```python
from build123d import *

# Parameters (mm, degrees)
BASEHEAD_DEPTH = 10.18
SKETCH5_R      = 8
BASEBODY_DEPTH = 35
CHAMFER1_SIZE  = 0.8


with BuildPart() as part:
    # Sketch2 → BaseHead (new body)
    with BuildSketch(Plane(origin=(0, 0, 0), x_dir=(0, 0, -1), z_dir=(1, 0, 0))):
        Polygon((11.835, -6.832940436), (11.835, 6.832940436), (0, 13.665880872), (-11.835, 6.832940436), (-11.835, -6.832940436), (0, -13.665880872), align=None)
    extrude(amount=BASEHEAD_DEPTH)

    # Sketch3 → BearingFace (revolve, cut)
    with BuildSketch(Plane.XY, mode=Mode.PRIVATE) as bearingface_sk:
        Polygon((10.18, 13.665880872), (10.18, 11.245), (9.38, 12.045), (9.38, 13.665880872), align=None)
    revolve(bearingface_sk.sketch.rotate(Axis((-0.957090588, 0, 0), (1, 0, 0)), 90), axis=Axis((-0.957090588, 0, 0), (1, 0, 0)), mode=Mode.SUBTRACT)

    # Sketch4 → HeadChamfer (revolve, cut)
    with BuildSketch(Plane.XY):
        Polygon((0, 13.665880872), (0.66638614, 13.665880872), (0, 11.835), align=None)
    revolve(axis=Axis((-0.493528746, 0, 0), (1, 0, 0)), mode=Mode.SUBTRACT)

    # Sketch5 → BaseBody (add)
    with BuildSketch(Plane(origin=(10.18, 0, 0), x_dir=(0, 0, -1), z_dir=(1, 0, 0))):
        with Locations(Location((0, 0, 0), (0, 0, 180))):
            Circle(SKETCH5_R)
    extrude(amount=BASEBODY_DEPTH)

    # Chamfer1
    chamfer1_edges = [part.edges().sort_by_distance(p)[0] for p in [
        (45.18, 0, -8),
    ]]
    chamfer(chamfer1_edges, length=CHAMFER1_SIZE)


solid = part.part
```
Could you check a few things on this model? Use its own coordinates, in mm. A direction names the side the tool comes from. Give positions to 0.01 mm unless a question says otherwise; leave off trailing zeros. Loops run counter-clockwise (first coordinate to the right, second up) from the corner with the lowest first, then second, coordinate; pieces in that order, holes last. Notation, with made-up numbers: (1.25, 74.25) -> (10.25, 74.25) arc R17 ccw to (10.25, 102.25) -> close; hole circle Ø9 at (27, 85). An arc over 180 degrees is marked (long way). Put each result on its own line as item: value.
(1) I'm going to push flat-ended pins straight in: pin 1 Ø4 at (y, z) = (9, 4.5) entering from +X; pin 2 Ø3 at (x, y) = (20, 5.5) entering from +Z; pin 3 Ø5 at (x, z) = (12, 6) entering from -Y. Where does each tip first touch, or does it pass through?
Computed:
pin 1: x = 10.18
pin 2: z = 6.93
pin 3: y = -10.6
(2) Please list where these lines run through material, in increasing order: probe 1 along X at (y, z) = (-8.25, 2.75); probe 2 along Z at (x, y) = (42, -1.5); probe 3 along Y at (x, z) = (13, -0.75). Write a range as [from, to].
Computed:
probe 1: [0, 10.18]
probe 2: [-7.86, 7.86]
probe 3: [-7.96, 7.96]
(3) Imagine slicing it at A-A on x = 16. Write out the boundary of the cut face in (y, z), plus the area to 3 significant figures.
Computed:
outline: circle Ø16 at (0, 0)
area: 201 mm^2
(4) For faces 1 (the face through (10.18, 8, -2)), 2 (the face through (9.38, 6, -11)), 3 (the face through (9.38, 6, 11)), which set-ups out of +Z, -Z, +X, -X, +Y, -Y let a thin tool reach every point of the face, with its end or its side?
Computed:
face 1: +X
face 2: -Z, +X, +Y
face 3: +Z, +X, +Y
